The listing builds one solid part. Answer for the finished solid, in the listing's coordinates (mm). A direction names the side the tool comes from. Round coordinates to 2 decimals unless told otherwise and drop trailing zeros. Loops run counter-clockwise (first coordinate to the right, second up) from the corner with the lowest first, then second, coordinate; pieces in that order, holes last. Notation, with made-up numbers: (59, 44) - (80, 44) arc R26 cw to (80, 66) - close; hole circle Ø2 at (14.5, 68.25). An arc over 180 degrees is marked (long way). Write item = value, one per line. Start each with the question number.
1) Given pin 1 Ø3 at (x, y) = (-15.5, -5) entering from -Z; pin 2 Ø3 at (x, z) = (135, -3) entering from -Y; pin 3 Ø5 at (x, z) = (-49.5, -4.5) entering from -Y, each flat-ended and moving along its own axis, determine where each tip first touches the part or whether it passes through.
2) Section A-A, the plane y = -3 is taken. Determine the outline of the cut face in (x, z).
3) A tool of negligible diameter and unlimited length cuts with its end or side. For faces 1 (the flat face through (178.5, -5, -2)), 2 (the cylindrical face through (-181, 0, 5)), 3 (the flat face through (-183.5, 0, 0)), from which of +Z, -Z, +X, -X, +Y, -Y can it reach the whole face along a straight path? Write none if from no direction.
4) Section B-B, the plane x = -82.5 is taken. Determine the outline of the cut face in (y, z), and give its area (3 significant figures).
5) Straight lines are drawn through the part: line 1 along X through (y, z) = (-5.5, 3); line 2 along Z through (x, y) = (83.5, 0.5); line 3 along Z through (x, y) = (9.5, 5.75). For each, find the intervals that lie inside material, in ascending order.
from build123d import *

# Parameters (mm, degrees)
SKETCH1_R           = 6.5
BOSS_EXTRUDE1_DEPTH = 178.5
SKETCH2_R           = 5
BOSS_EXTRUDE2_DEPTH = 5
BOSS_EXTRUDE3_START = 5
SKETCH3_R           = 5
BOSS_EXTRUDE3_DEPTH = 5


with BuildPart() as part:
    # Sketch1 → Boss-Extrude1 (new, symmetric)
    with BuildSketch(Plane(origin=(0, 0, 0), x_dir=(0, 0, -1), z_dir=(1, 0, 0))):
        Circle(SKETCH1_R)
    extrude(amount=BOSS_EXTRUDE1_DEPTH, both=True)

    # Sketch2 → Boss-Extrude2 (add)
    with BuildSketch(Plane(origin=(178.5, 0, 0), x_dir=(0, 0, -1), z_dir=(1, 0, 0))):
        Circle(SKETCH2_R)
    extrude(amount=BOSS_EXTRUDE2_DEPTH)

    # Sketch3 → Boss-Extrude3 (add)
    with BuildSketch(Plane.ZY.offset(178.5).offset(BOSS_EXTRUDE3_START)):
        with Locations(Location((0, 0, 0), (0, 0, 180))):
            Circle(SKETCH3_R)
    extrude(amount=-BOSS_EXTRUDE3_DEPTH)


solid = part.part
Geometry check:
q1.pin_1 = -5.48
q1.pin_2 = -6.32
q1.pin_3 = -6.18
q2.outline = (-183.5, -4) - (-178.5, -4) - (-178.5, -5.77) - (178.5, -5.77) - (178.5, -4) - (183.5, -4) - (183.5, 4) - (178.5, 4) - (178.5, 5.77) - (-178.5, 5.77) - (-178.5, 4) - (-183.5, 4) - close
q3.face_1 = +X
q3.face_2 = -X
q3.face_3 = +Z, -Z, -X, +Y, -Y
q4.outline = circle Ø13 at (0, 0)
q4.area = 133 mm2
q5.line_1 = -178.5 to 178.5
q5.line_2 = -6.48 to 6.48
q5.line_3 = -3.03 to 3.03
